Model file for the job. Use its own axes, mm. Coordinates: 2 decimals unless noted, no trailing zeros. Order: outer loops, then holes, each group sorted by start corner. A loop starts at its lowest first (then second) coordinate and runs counter-clockwise, first axis right, second up. Notation, with made-up numbers: (3, 30.25) -> (48, 30.25) arc R17 cw to (48, 45.25) -> close; hole circle Ø10 at (-17, -21.5). An arc over 180 degrees is marked (long way). Use CSV: the item, a comma, the result in double quotes. Start each with the question number.
(1) Cut at A-A on y = 364.5. Write the cut outline in (x, z), plus the area to 3 significant figures.
(2) Pin check, flat tips, straight feed: pin 1 Ø1.5 at (y, z) = (282.5, -9.5) entering from -X; pin 2 Ø0.9 at (x, y) = (3, 143.5) entering from +Z; pin 3 Ø1.6 at (x, y) = (10.5, 410) entering from +Z; pin 4 Ø4 at (y, z) = (109.5, -6.5) entering from +X. Stop position of each tip, or through.
(3) Probe L1, parallel to Y at x = 10, z = -2.7; L2, parallel to Z at x = 17.5, y = 397.5; L3, parallel to X at y = 410, z = -1.6. List the from-to ranges inside material, lowest first.
```python
from build123d import *

# Parameters (mm, degrees)
BOSS_EXTRUDE1_DEPTH = 435
SKETCH2_R           = 2.75
CUT_EXTRUDE1_DEPTH  = 5


with BuildPart() as part:
    # Sketch1 → Boss-Extrude1 (new body)
    with BuildSketch(Plane(origin=(0, 0, 0), x_dir=(1, 0, 0), z_dir=(0, 1, 0))):
        Polygon((0, 0), (20, 0), (20, 3), (15, 3), (15, 8), (18, 8), (18, 11), (2, 11), (2, 8), (5, 8), (5, 3), (0, 3), align=None)
    extrude(amount=BOSS_EXTRUDE1_DEPTH)

    # Sketch2 → Cut-Extrude1 (cut)
    with BuildSketch(Plane.XY):
        with Locations((10, 410)):
            Circle(SKETCH2_R)
        with Locations((10, 25)):
            Circle(SKETCH2_R)
    extrude(amount=-CUT_EXTRUDE1_DEPTH, mode=Mode.SUBTRACT)


solid = part.part
```
Outcome:
1,outline,"(0, -3) -> (5, -3) -> (5, -8) -> (2, -8) -> (2, -11) -> (18, -11) -> (18, -8) -> (15, -8) -> (15, -3) -> (20, -3) -> (20, 0) -> (0, 0) -> close"
1,area,"158 mm2"
2,pin 1,"x = 2"
2,pin 2,"z = 0"
2,pin 3,"z = -5"
2,pin 4,"x = 18"
3,L1,"0 to 22.25, 27.75 to 407.25, 412.75 to 435"
3,L2,"-11 to -8, -3 to 0"
3,L3,"0 to 7.25, 12.75 to 20"
